The model under review builds one solid part; all positions refer to its coordinate system, in mm. A direction names the side the tool comes from. Round coordinates to 2 decimals unless told otherwise and drop trailing zeros. Order: outer loops, then holes, each group sorted by start corner. A loop starts at its lowest first (then second) coordinate and runs counter-clockwise, first axis right, second up. Notation, with made-up numbers: (-4.5, -34) - (42.5, -34) arc R17 cw to (42.5, -19) - close; hole circle Ø9 at (70, -26). An arc over 180 degrees is marked (long way). One line per question, with ' | ' between items. Start each with the question number.
Item 1: For L1, parallel to X at y = 19.5, z = 1.2; L2, parallel to Y at x = 19.5, z = 0.3; L3, parallel to X at y = 17, z = 4.15, list the stretches that pass through material, from the lowest coordinate up. Write a range as [from, to].
Item 2: Add section B-B on z = 0.95. State the section outline as (x, y) points.
Item 3: Draft analysis for pull direction Y (two halves, no side actions). For faces 3 (the face through (13, 15.75, 2)), 4 (the face through (12, 21.25, 2)), 5 (the face through (0, 18, 2)), 6 (the face through (59, 37, 2)), state which applies: +Y half, -Y half, draft (parallel to the pull), parting line (faces both ways), or undercut.
Item 4: Insertion check: pin 1 Ø2.5 at (x, z) = (9.5, 1.5) entering from -Y. The pin has a flat end and moves straight along its axis. Give the tip position at first contact, or say it passes through.
Item 5: Add section A-A on y = 18.5. State the section outline as (x, z) points.
Item 6: Tool access review of faces 1 (the face through (59, 19, 0)), 2 (the face through (107, 21.25, 2)): name each direction out of +Z, -Z, +X, -X, +Y, -Y from which nothing blocks a thin tool from reaching the whole face with its end or side.
from build123d import *

# Parameters (mm, degrees)
SKETCH_1_W      = 120
SKETCH_1_H      = 37
EXTRUDE_1_DEPTH = 5


with BuildPart() as part:
    # 草图1 → 凸台-拉伸1 (new body)
    with BuildSketch(Plane.XY):
        with Locations((60, 18.5)):
            Rectangle(SKETCH_1_W, SKETCH_1_H)
        with BuildLine():
            Line((5, 21.25), (20, 21.25))
            ThreePointArc((20, 21.25), (22.75, 18.5), (20, 15.75))
            Line((20, 15.75), (5, 15.75))
            ThreePointArc((5, 15.75), (2.25, 18.5), (5, 21.25))
        make_face(mode=Mode.SUBTRACT)
        with BuildLine():
            Line((115, 15.75), (100, 15.75))
            ThreePointArc((100, 15.75), (97.25, 18.5), (100, 21.25))
            Line((100, 21.25), (115, 21.25))
            ThreePointArc((115, 21.25), (117.75, 18.5), (115, 15.75))
        make_face(mode=Mode.SUBTRACT)
    extrude(amount=EXTRUDE_1_DEPTH)


solid = part.part
Determined:
1) L1: [0, 2.44], [22.56, 97.44], [117.56, 120] | L2: [0, 15.75], [21.25, 37] | L3: [0, 2.7], [22.3, 97.7], [117.3, 120]
2) outline: (0, 0) - (120, 0) - (120, 37) - (0, 37) - close; hole (5, 15.75) - (20, 15.75) arc R2.75 ccw to (20, 21.25) - (5, 21.25) arc R2.75 ccw to start; hole (100, 15.75) - (115, 15.75) arc R2.75 ccw to (115, 21.25) - (100, 21.25) arc R2.75 ccw to start
3) face 3: undercut | face 4: undercut | face 5: draft | face 6: +Y half
4) pin 1: y = 0
5) outline: (0, 0) - (2.25, 0) - (2.25, 5) - (0, 5) - close; (22.75, 0) - (97.25, 0) - (97.25, 5) - (22.75, 5) - close; (117.75, 0) - (120, 0) - (120, 5) - (117.75, 5) - close
6) face 1: -Z, +X, -X, +Y, -Y | face 2: +Z, -Z
